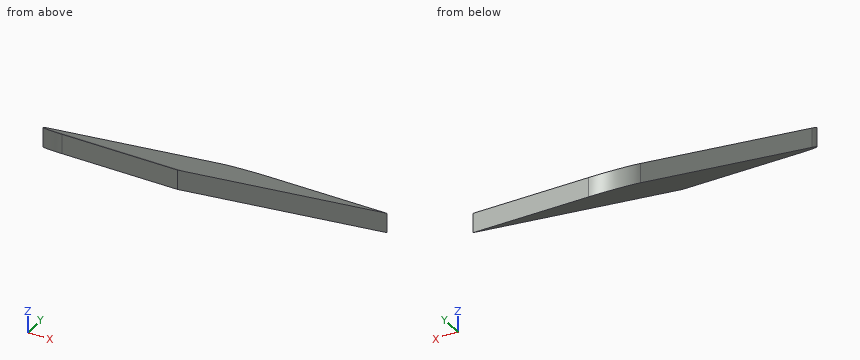
```python
from build123d import *

# Parameters (mm, degrees)
EXTRUDE_2_DEPTH     = 100
SKETCH_3_OUTSIDE_W  = 133.064
SKETCH_3_OUTSIDE_H  = 143.064
CUT_EXTRUDE_5_DEPTH = 100


with BuildPart() as part:
    # 草图1 → 凸台-拉伸2 (new body)
    with BuildSketch(Plane.XY):
        with BuildLine():
            Line((-679.821296296, 67.7), (-679.821296296, -42.3))
            Line((-679.821296296, -42.3), (-714.821296296, -42.3))
            ThreePointArc((-714.821296296, -42.3), (-721.892364108, -39.371067812), (-724.821296296, -32.3))
            Line((-724.821296296, -32.3), (-724.821296296, 57.7))
            ThreePointArc((-724.821296296, 57.7), (-721.892364108, 64.771067812), (-714.821296296, 67.7))
            Line((-714.821296296, 67.7), (-679.821296296, 67.7))
        make_face()
    extrude(amount=EXTRUDE_2_DEPTH)

    # 草图3 outside → 切除-拉伸5 (cut)
    with BuildSketch(Plane(origin=(-679.821296296, 0, 0), x_dir=(0, 0, -1), z_dir=(1, 0, 0))):
        with Locations((-50, 12.7)):
            Rectangle(SKETCH_3_OUTSIDE_W, SKETCH_3_OUTSIDE_H)
        Polygon((-86.021487915, -42.3), (-80, -42.3), (-6.182486595, 67.7), (-12.203974509, 67.7), (-84.151797754, -39.513860124), align=None, mode=Mode.SUBTRACT)
    extrude(amount=-CUT_EXTRUDE_5_DEPTH, mode=Mode.SUBTRACT)


solid = part.part
```
Geometry: final body of the model. Coordinates: model frame, mm. Coordinates: 2 decimals unless noted, no trailing zeros. Order: outer loops, then holes, each group sorted by start corner. A loop starts at its lowest first (then second) coordinate and runs counter-clockwise, first axis right, second up. Notation, with made-up numbers: M 69.25,-35 L 115.25,-35 A35 ccw 115.25,0 Z; hole C -16.5,88.25 d11. An arc over 180 degrees is marked long. Answer in a Markdown table with one row per item. Add a question column.
Q1. Line query: L1, parallel to Z at x = -721, y = 22.5; L2, parallel to Z at x = -683, y = 12; L3, parallel to Y at x = -703.5, z = 48.5. Output: solid intervals per line, ascending.
Q2. Section query D-D on z = 31. Return the cut outline in (x, y).
Q3. Section query A-A on x = -693. Return the cut outline in (y, z).
Q4. Contact query for flat-ended pins moving along their axis: P1, Ø5, axis at x = -700, y = 19.5, coming from the -Z side; P2, Ø12, axis at x = -689.5, z = 31, coming from the +Y side; P3, Ø1.5, axis at x = -684.5, y = 36, coming from the +Z side. Output: stop coordinate, or through.
Q5. Section query C-C on y = 61. Return the cut outline in (x, z).
Q6. Section query B-B on z = 15. Return the cut outline in (x, y).
Completed:
| question | item | result |
|---|---|---|
| 1 | L1 | z = 36.51 to 42.54 |
| 1 | L2 | z = 43.56 to 49.58 |
| 1 | L3 | y = 4.64 to 13.61 |
| 2 | outline | M -724.82,30.72 L -679.82,30.72 L -679.82,39.69 L -724.82,39.69 Z |
| 3 | outline | M -42.3,80 L 67.7,6.18 L 67.7,12.2 L -42.3,86.02 Z |
| 4 | P1 | stops at z = 36.85 |
| 4 | P2 | stops at y = 48.63 |
| 4 | P3 | stops at z = 33.98 |
| 5 | outline | M -724.26,10.68 L -679.82,10.68 L -679.82,16.7 L -724.26,16.7 Z |
| 6 | outline | M -724.82,54.56 L -679.82,54.56 L -679.82,63.53 L -722.94,63.53 A10 ccw -724.82,57.7 Z |
